```python
from build123d import *

# Parameters (mm, degrees)
BASE_PLATE_DEPTH              = 12
BASE_HOLE_DEPTH               = 12
UPRIGHT_BLOCK_SKETCH_W        = 42
UPRIGHT_BLOCK_SKETCH_H        = 12
UPRIGHT_BLOCK_DEPTH           = 60
CLEVIS_EAR_DEPTH              = 7.5
CLEVIS_EAR_EXTENSION_SKETCH_W = 45
CLEVIS_EAR_EXTENSION_SKETCH_H = 40
CLEVIS_EAR_EXTENSION_DEPTH    = 7.5
CLEVIS_PIN_BORE_SKETCH_R      = 9
CLEVIS_PIN_BORE_DEPTH         = 90.5
SADDLE_BLOCK_SKETCH_W         = 12
SADDLE_BLOCK_SKETCH_H         = 13
SADDLE_BLOCK_DEPTH            = 60
SADDLE_CUT_SKETCH_R           = 13
SADDLE_CUT_DEPTH              = 12
THROUGH_HOLE_A_SKETCH_R       = 9
THROUGH_HOLE_A_DEPTH          = 139
THROUGH_HOLE_B_SKETCH_R       = 5
THROUGH_HOLE_B_DEPTH          = 139
THROUGH_HOLE_C_SKETCH_R       = 8
THROUGH_HOLE_C_DEPTH          = 139


with BuildPart() as part:
    # Base Plate Sketch → Base Plate (new body)
    with BuildSketch(Plane(origin=(0, 0, 0), x_dir=(1, 0, 0), z_dir=(0, 1, 0))):
        Polygon((0, 0), (30, 0), (30, 100), (-30, 100), (-30, 0), align=None)
    extrude(amount=BASE_PLATE_DEPTH)

    # Base Hole Sketch → Base Hole (cut)
    with BuildSketch(Plane(origin=(0, 12, 0), x_dir=(1, 0, 0), z_dir=(0, 1, 0))):
        with BuildLine():
            ThreePointArc((1.57e-07, 0), (-21.21320338, 8.786796509), (-30, 30))
            Line((-30, 30), (-30, 0))
            Line((-30, 0), (1.57e-07, 0))
        make_face()
        with BuildLine():
            Line((30, 0), (30, 30))
            ThreePointArc((30, 30), (21.213203491, 8.78679662), (1.57e-07, 0))
            Line((1.57e-07, 0), (30, 0))
        make_face()
    extrude(amount=-BASE_HOLE_DEPTH, mode=Mode.SUBTRACT)

    # Upright Block Sketch → Upright Block (add)
    with BuildSketch(Plane(origin=(30, 0, 0), x_dir=(0, 0, -1), z_dir=(1, 0, 0))):
        Polygon((50, 12), (92, 12), (92, 25), (62, 25), (50, 25), align=None)
        with Locations((71, 6)):
            Rectangle(UPRIGHT_BLOCK_SKETCH_W, UPRIGHT_BLOCK_SKETCH_H)
    extrude(amount=-UPRIGHT_BLOCK_DEPTH)

    # Clevis Ear Sketch → Clevis Ear (add)
    with BuildSketch(Plane.ZY.offset(30)):
        with BuildLine():
            Line((-51, 55), (-51, 25))
            Line((-51, 25), (-91, 25))
            Line((-91, 25), (-91, 55))
            ThreePointArc((-91, 55), (-71, 75), (-51, 55))
        make_face()
    clevis_ear = extrude(amount=-CLEVIS_EAR_DEPTH)

    # Clevis Ear Mirror: Clevis Ear across plane
    add(clevis_ear.mirror(Plane(origin=(0, 0, 0), x_dir=(0, 0, 1), z_dir=(1, 0, 0))))

    # Clevis Ear Extension Sketch → Clevis Ear Extension (add)
    with BuildSketch(Plane(origin=(0, 25, 0), x_dir=(1, 0, 0), z_dir=(0, 1, 0))):
        with Locations((0, 71)):
            Rectangle(CLEVIS_EAR_EXTENSION_SKETCH_W, CLEVIS_EAR_EXTENSION_SKETCH_H)
    extrude(amount=CLEVIS_EAR_EXTENSION_DEPTH)

    # Clevis Pin Bore Sketch → Clevis Pin Bore (cut)
    with BuildSketch(Plane(origin=(0, 32.5, 0), x_dir=(1, 0, 0), z_dir=(0, 1, 0))):
        with Locations(Location((0, 71, 0), (0, 0, 270))):
            Circle(CLEVIS_PIN_BORE_SKETCH_R)
    extrude(amount=-CLEVIS_PIN_BORE_DEPTH, mode=Mode.SUBTRACT)

    # Saddle Block Sketch → Saddle Block (add)
    with BuildSketch(Plane(origin=(30, 0, 0), x_dir=(0, 0, -1), z_dir=(1, 0, 0))):
        with Locations((44, 18.5)):
            Rectangle(SADDLE_BLOCK_SKETCH_W, SADDLE_BLOCK_SKETCH_H)
    extrude(amount=-SADDLE_BLOCK_DEPTH)

    # Saddle Cut Sketch → Saddle Cut (cut)
    with BuildSketch(Plane.XY.offset(-38)):
        with Locations((0, 25)):
            Circle(SADDLE_CUT_SKETCH_R)
    extrude(amount=-SADDLE_CUT_DEPTH, mode=Mode.SUBTRACT)

    # Through Hole A Sketch → Through Hole A (cut)
    with BuildSketch(Plane.ZY.offset(30)):
        with Locations((-71, 55)):
            Circle(THROUGH_HOLE_A_SKETCH_R)
    extrude(amount=-THROUGH_HOLE_A_DEPTH, mode=Mode.SUBTRACT)

    # Through Hole B Sketch → Through Hole B (cut)
    with BuildSketch(Plane.ZY.offset(30)):
        with Locations((-66, 12)):
            Circle(THROUGH_HOLE_B_SKETCH_R)
    extrude(amount=-THROUGH_HOLE_B_DEPTH, mode=Mode.SUBTRACT)

    # Through Hole C Sketch → Through Hole C (cut)
    with BuildSketch(Plane(origin=(0, 12, 0), x_dir=(1, 0, 0), z_dir=(0, 1, 0))):
        with Locations(Location((0, 18, 0), (0, 0, 270))):
            Circle(THROUGH_HOLE_C_SKETCH_R)
    extrude(amount=-THROUGH_HOLE_C_DEPTH, mode=Mode.SUBTRACT)


solid = part.part
```
Verification items for the finished model (mm, model axes). A direction names the side the tool comes from. Give positions to 0.01 mm unless a question says otherwise; leave off trailing zeros. Order: outer loops, then holes, each group sorted by start corner. A loop starts at its lowest first (then second) coordinate and runs counter-clockwise, first axis right, second up. Notation, with made-up numbers: M 43.25,42.25 L 58.25,42.25 A32 ccw 58.25,73.25 Z; hole C 27,-5 d7. An arc over 180 degrees is marked long. Return JSON: item names as keys, results as strings. Group by question number.
1) Section check D-D on x = 3. Record the cut outline in (y, z), and give its area (3 significant figures).
2) Section check A-A on y = 39.5. Record the cut outline in (x, z).
3) Section check B-B on z = -59. Record the cut outline in (x, y).
4) Go/stop test with flat-tipped pins: pin 1 Ø0.5 at (x, z) = (1.5, -91.5) entering from +Y; pin 2 Ø2.5 at (x, z) = (-7, -95) entering from +Y; pin 3 Ø6.5 at (x, y) = (18.5, 17.5) entering from +Z. Record where each tip stops, or that it passes through.
5) Scan lines: line 1 (X direction, y = 62, z = -81.5); line 2 (Z direction, x = 6, y = 6); line 3 (Y direction, x = 5, z = -43). Record each from-to range of solid material in increasing order.
6) Section check C-C on z = -74. Record the cut outline in (x, y), and give its area (3 significant figures).
7) Mould release check, pull along X, two halves, no side actions. Record for faces 5 (the face through (-22.5, 45, -71)), 6 (the face through (0, 0, -49)), 7 (the face through (30, 30, -72)): pulls with the +X half, pulls with the -X half, needs draft (parallel to the pull), parting line crosses it, or undercut.
8) Access from +Z, -Z, +X, -X, +Y, -Y to the whole of each face (thin tool, end or side, straight path). Record for faces 1 (the face through (0.4, 25, -50.2)), 2 (the face through (0, 20, -50)), 3 (the face through (-0.3, 32.5, -80.2)), 4 (the face through (0, 18, -92)).
Answer block:
{
 "1": {"outline": "M 0,-100 L 12,-100 L 12,-92 L 25,-92 L 25,-91 L 32.5,-91 L 32.5,-79.49 L 0,-79.49 Z; M 0,-62.51 L 8.41,-62.51 A5 cw 15.59,-62.51 L 32.5,-62.51 L 32.5,-51 L 25,-51 L 25,-50 L 12.35,-50 L 12.35,-38 L 12,-38 L 12,-25.42 L 0,-25.42 Z; M 0,-10.58 L 12,-10.58 L 12,-0.15 L 0,-0.15 Z", "area": "1,310 mm^2"},
 "2": {"outline": "M -30,-91 L -22.5,-91 L -22.5,-51 L -30,-51 Z; M 22.5,-91 L 30,-91 L 30,-51 L 22.5,-51 Z"},
 "3": {"outline": "M -30,0 L 30,0 L 30,71 L 22.5,71 L 22.5,32.5 L -22.5,32.5 L -22.5,71 L -30,71 Z"},
 "4": {"pin 1": "stops at y = 25", "pin 2": "stops at y = 12", "pin 3": "stops at z = -38"},
 "5": {"line 1": "x = -30 to -22.5, 22.5 to 30", "line 2": "z = -100 to -77.71, -64.29 to -23.29, -12.71 to -0.61", "line 3": "y = 0 to 13"},
 "6": {"outline": "M -30,0 L -8.49,0 L -8.49,32.5 L -22.5,32.5 L -22.5,46.51 L -30,46.51 Z; M -30,63.49 L -22.5,63.49 L -22.5,74.77 L -30,74.77 Z; M 8.49,0 L 30,0 L 30,46.51 L 22.5,46.51 L 22.5,32.5 L 8.49,32.5 Z; M 22.5,63.49 L 30,63.49 L 30,74.77 L 22.5,74.77 Z", "area": "1,780 mm^2"},
 "7": {"face 5": "undercut", "face 6": "needs draft", "face 7": "pulls with the +X half"},
 "8": {"face 1": "+Z, +X, -X, +Y", "face 2": "+Z, +Y", "face 3": "+Z, -Z, +Y", "face 4": "-Z, +X, -X, +Y"}
}
